Can you work these out from the model? Positions are in its coordinate system, mm. Give positions to 0.01 mm unless a question says otherwise; leave off trailing zeros. Order: outer loops, then holes, each group sorted by start corner. A loop starts at its lowest first (then second) coordinate and runs counter-clockwise, first axis right, second up.
```python
from build123d import *

# Parameters (mm, degrees)
SKETCH1_W               = 1630
SKETCH1_H               = 415
BOSS_EXTRUDE1_DEPTH     = 25
CHAMFER1_SIZE           = 20
CUT_EXTRUDE1_DEPTH      = 842.371647965
CUT_EXTRUDE1_DEPTH_BACK = 842.371647965
SKETCH2_R               = 20
SKETCH2_W               = 1000
SKETCH2_H               = 200


with BuildPart() as part:
    # Sketch1 → Boss-Extrude1 (new body)
    with BuildSketch(Plane.XY):
        Rectangle(SKETCH1_W, SKETCH1_H)
    extrude(amount=BOSS_EXTRUDE1_DEPTH)

    # Chamfer1
    chamfer1_edges = [part.edges().sort_by_distance(p)[0] for p in [
        (-815, 207.5, 12.5),
        (815, 207.5, 12.5),
        (815, -207.5, 12.5),
        (-815, -207.5, 12.5),
    ]]
    chamfer(chamfer1_edges, length=CHAMFER1_SIZE)

    # Sketch2 → Cut-Extrude1 (cut, two sides: drawn at the far end of the back side and taken through both)
    with BuildSketch(Plane.XY.offset(25).offset(-CUT_EXTRUDE1_DEPTH_BACK)):
        with Locations((-765, 127.5)):
            Circle(SKETCH2_R)
        with Locations((765, 127.5)):
            Circle(SKETCH2_R)
        with Locations((155, 142.5)):
            Rectangle(SKETCH2_W, SKETCH2_H)
    extrude(amount=CUT_EXTRUDE1_DEPTH + CUT_EXTRUDE1_DEPTH_BACK, mode=Mode.SUBTRACT)


solid = part.part
```
1) Suppose I cut it at C-C (y = 127.5). Please give me the cut outline in (x, z).
2) Suppose I cut it at B-B (z = 15.5). Please give me the cut outline in (x, y), and give its area (3 significant figures).
3) Suppose I cut it at A-A (x = -765). Please give me the cut outline in (y, z).
4) If I drill on line 1 (X direction, y = 127.5, z = 17.25); line 2 (Y direction, x = -765, z = 15); line 3 (Y direction, x = -231.5, z = 5.75), over which ranges is the centre line in solid material (lowest first)?
5) I'm going to push a flat-ended pin straight in: pin 1 Ø4 at (x, z) = (103.5, 15.5) entering from +Y. Where does the tip first touch, or does it pass through?
6) We'd pull the mould along Y, two halves only. Please class faces 1 (the face through (-780.87, 115.33, 12.33)), 2 (the face through (-11, -43, 0)): +Y half, -Y half, draft (parallel to the pull), parting line (faces both ways), or undercut.
7) Suppose I cut it at D-D (x = -52.5). Please give me the cut outline in (y, z).
Results:
1. outline: (-815, 0) - (-785, 0) - (-785, 25) - (-815, 25) - close; (-745, 0) - (-345, 0) - (-345, 25) - (-745, 25) - close; (655, 0) - (745, 0) - (745, 25) - (655, 25) - close; (785, 0) - (815, 0) - (815, 25) - (785, 25) - close
2. outline: (-815, -187.5) - (-795, -207.5) - (795, -207.5) - (815, -187.5) - (815, 187.5) - (795, 207.5) - (655, 207.5) - (655, 42.5) - (-345, 42.5) - (-345, 207.5) - (-795, 207.5) - (-815, 187.5) - close; hole circle Ø40 at (-765, 127.5); hole circle Ø40 at (765, 127.5)
2. area: 508,000 mm2
3. outline: (-207.5, 0) - (107.5, 0) - (107.5, 25) - (-207.5, 25) - close; (147.5, 0) - (207.5, 0) - (207.5, 25) - (147.5, 25) - close
4. line 1: x = -815 to -785, -745 to -345, 655 to 745, 785 to 815
4. line 2: y = -207.5 to 107.5, 147.5 to 207.5
4. line 3: y = -207.5 to 42.5
5. pin 1: stops at y = 42.5
6. face 1: undercut
6. face 2: draft
7. outline: (-207.5, 0) - (42.5, 0) - (42.5, 25) - (-207.5, 25) - close
